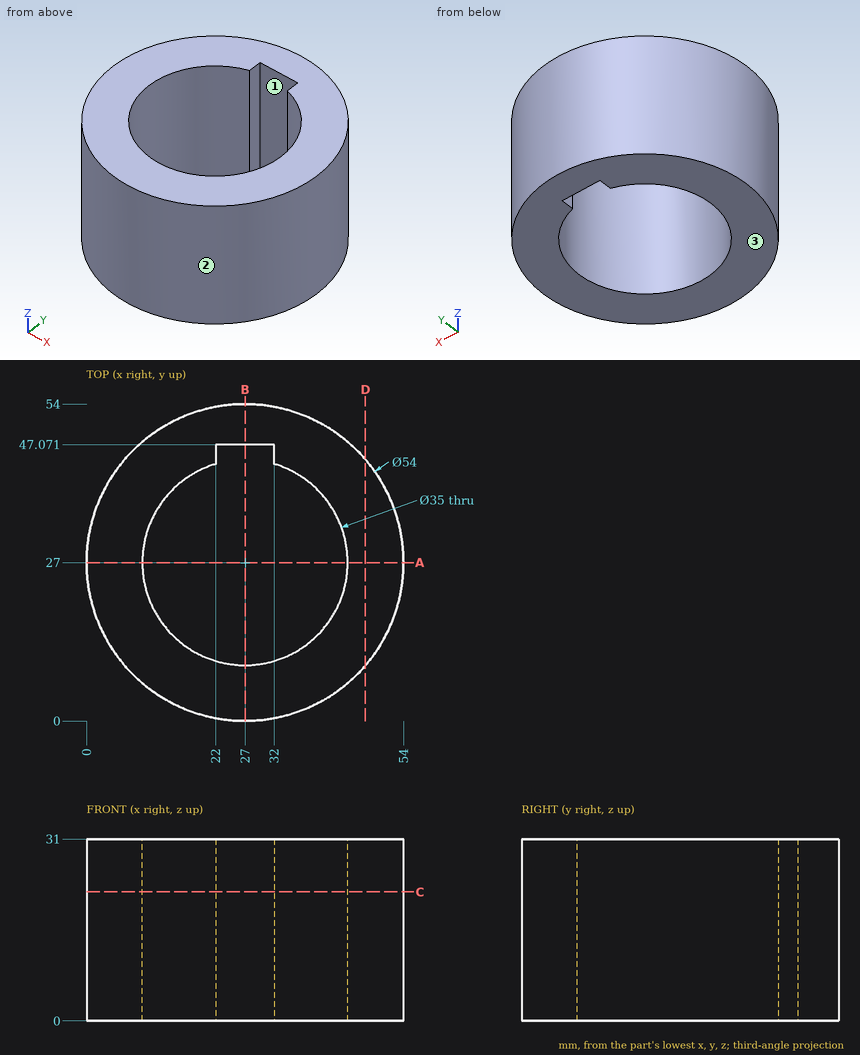
Verification items for this drawing (mm, ordinates from the low corner). Round coordinates to 2 decimals unless told otherwise and drop trailing zeros. Loops run counter-clockwise (first coordinate to the right, second up) from the corner with the lowest first, then second, coordinate; pieces in that order, holes last. Notation, with made-up numbers: (-32.5, 41.5) - (-5.5, 41.5) arc R30 ccw to (-5.5, 69.5) - close; hole circle Ø4 at (-11, 22.5). An arc over 180 degrees is marked (long way). Answer as CSV lines item,"result". Start each with the question number.
Item 1: Section check D-D (x = 47.5). Record the boundary of the cut face in (y, z), and give its area (3 significant figures).
Item 2: Section check B-B (x = 27). Record the boundary of the cut face in (y, z).
Item 3: Section check C-C (z = 22). Record the boundary of the cut face in (x, y), and give its area (3 significant figures).
Item 4: Section check A-A (y = 27). Record the boundary of the cut face in (x, z).
Item 5: Scan lines: line 1 (X direction, y = 27, z = 10); line 2 (Y direction, x = 27, z = 20); line 3 (X direction, y = 29.5, z = 13) (1 decimal). Record each from-to range of solid material in increasing order. Write a range as [from, to].
Item 6: Depth check by flat-ended pin: P1, Ø21, axis at x = 27, y = 27, coming from the -Z side; P2, Ø2, axis at x = 33, z = 25, coming from the +Y side; P3, Ø5, axis at x = 47, z = 14.5, coming from the +Y side; P4, Ø12, axis at x = 45, z = 12, coming from the -Y side. Enter the tip coordinate at first touch or a pass-through.
Item 7: Release check for a two-part mould opening along Y. For the marked faces 1, 2 and 3 record: +Y half, -Y half, draft (parallel to the pull), parting line (faces both ways), or undercut.
Report:
1,outline,"(9.43, 0) - (44.57, 0) - (44.57, 31) - (9.43, 31) - close"
1,area,"1,090 mm2"
2,outline,"(0, 0) - (9.5, 0) - (9.5, 31) - (0, 31) - close; (47.07, 0) - (54, 0) - (54, 31) - (47.07, 31) - close"
3,outline,"circle Ø54 at (27, 27); hole (22, 43.77) arc R17.5 ccw (long way) to (32, 43.77) - (32, 47.07) - (22, 47.07) - close"
3,area,"1,300 mm2"
4,outline,"(0, 0) - (9.5, 0) - (9.5, 31) - (0, 31) - close; (44.5, 0) - (54, 0) - (54, 31) - (44.5, 31) - close"
5,line 1,"x = [0, 9.5], [44.5, 54]"
5,line 2,"y = [0, 9.5], [47.07, 54]"
5,line 3,"x = [0.1, 9.7], [44.3, 53.9]"
6,P1,"passes through"
6,P2,"stops at y = 53.53"
6,P3,"stops at y = 47.56"
6,P4,"stops at y = 2.81"
7,face 1,"undercut"
7,face 2,"parting line"
7,face 3,"draft"
